Geometry check sheet. Reference: the model listing, model coordinates, mm. A direction names the side the tool comes from. Give positions to 0.01 mm unless a question says otherwise; leave off trailing zeros. Loops run counter-clockwise (first coordinate to the right, second up) from the corner with the lowest first, then second, coordinate; pieces in that order, holes last.
1. Cross-section at B-B, the plane x = 8.5. Record the cut outline in (y, z), plus the area to 3 significant figures.
2. Cross-section at C-C, the plane y = 48.5. Record the cut outline in (x, z).
3. Release check for a two-part mould opening along Z. For faces 1 (the flat face through (-1, 2, 67.5)), 2 (the flat face through (1, 0, 1)), 3 (the cylindrical face through (-47.165, -5.07, -41.506)) record: +Z half, -Z half, draft (parallel to the pull), parting line (faces both ways), or undercut.
4. Cross-section at D-D, the plane z = 47.5. Record the cut outline in (x, y).
5. Go/stop test with flat-tipped pins: pin 1 Ø10.5 at (x, z) = (-26, 17.5) entering from +Y; pin 2 Ø10 at (x, z) = (2.5, -49.5) entering from +Y; pin 3 Ø8 at (x, y) = (54.5, 7.5) entering from -Z; pin 4 Ø11 at (x, z) = (-47.43, 47.5) entering from -Y. Record where each tip stops, or that it passes through.
6. Tool access check on faces 4 (the flat face through (46, 3, -3)), 5 (the flat face through (-53, 0, -35)), 6 (the flat face through (-3, 26, -5)), 7 (the flat face through (27.643, -5, 1)), 8 (the flat face through (20, 10, 21)). Record the directions out of +Z, -Z, +X, -X, +Y, -Y that give a thin tool (end or side, any length) a straight path to the whole face; none if there is none.
7. Cross-section at A-A, the plane z = -47.5. Record the cut outline in (x, y).
8. Material ranges on L1, parallel to X at y = -4, z = -47; L2, parallel to X at y = 58, z = -33; L3, parallel to Y at x = 38, z = -35, recorded low to high.
from build123d import *

# Parameters (mm, degrees)
BASE_PLATE_SKETCH_W     = 135
BASE_PLATE_SKETCH_H     = 20
BASE_PLATE_DEPTH        = 67.5
BOTTOM_CHANNEL_DEPTH    = 152.265495074
TOP_RECESS_SKETCH_W     = 30
TOP_RECESS_SKETCH_H     = 10
TOP_RECESS_DEPTH        = 152.265495074
UPRIGHT_LUG_SKETCH_R    = 10
UPRIGHT_LUG_DEPTH       = 75
SIDE_GUSSET_DEPTH       = 3
CENTRE_START            = -37.5
CENTRE_RIB_DEPTH        = 3
MOUNTING_HOLES_SKETCH_R = 6
MOUNTING_HOLES_12_DEPTH = 128.818230312


with BuildPart() as part:
    # Base Plate Sketch → Base Plate (new, symmetric)
    with BuildSketch(Plane.XY):
        Rectangle(BASE_PLATE_SKETCH_W, BASE_PLATE_SKETCH_H)
    extrude(amount=BASE_PLATE_DEPTH, both=True)

    # Bottom Channel Sketch → Bottom Channel (cut, through all)
    with BuildSketch(Plane.XY.offset(67.5)):
        Polygon((27.643184154, 0), (0, 0), (-27.356815846, 0), (-27.356815846, -10), (27.643184154, -10), align=None)
    extrude(amount=-BOTTOM_CHANNEL_DEPTH, mode=Mode.SUBTRACT)

    # Top Recess Sketch → Top Recess (cut, through all)
    with BuildSketch(Plane.XY.offset(67.5)):
        with Locations((-52.5, 5)):
            Rectangle(TOP_RECESS_SKETCH_W, TOP_RECESS_SKETCH_H)
        with Locations((52.5, 5)):
            Rectangle(TOP_RECESS_SKETCH_W, TOP_RECESS_SKETCH_H)
    extrude(amount=-TOP_RECESS_DEPTH, mode=Mode.SUBTRACT)

    # Upright Lug Sketch → Upright Lug (add)
    with BuildSketch(Plane(origin=(37.5, 0, 0), x_dir=(0, 0, -1), z_dir=(1, 0, 0))):
        with BuildLine():
            Line((67.5, 10), (67.5, 55))
            ThreePointArc((67.5, 55), (47.5, 75), (27.5, 55))
            Line((27.5, 55), (27.5, 10))
            Line((27.5, 10), (67.5, 10))
        make_face()
        with Locations((47.5, 55)):
            Circle(UPRIGHT_LUG_SKETCH_R, mode=Mode.SUBTRACT)
    extrude(amount=-UPRIGHT_LUG_DEPTH)

    # Side Gusset Sketch → Side Gusset (add, symmetric)
    with BuildSketch(Plane.XY):
        Polygon((-67.5, 0), (-37.5, 10), (-37.5, 0), align=None)
    side_gusset = extrude(amount=SIDE_GUSSET_DEPTH, both=True)

    # Side Gusset Mirror: Side Gusset across plane
    add(side_gusset.mirror(Plane(origin=(0, 0, 0), x_dir=(0, 0, 1), z_dir=(1, 0, 0))))

    # Centre Rib Sketch → Centre Rib (add, symmetric)
    with BuildSketch(Plane(origin=(37.5, 0, 0), x_dir=(0, 0, -1), z_dir=(1, 0, 0)).offset(CENTRE_START)):
        Polygon((-67.5, 10), (35.500032612, 69.198001073), (35.500032612, 10), (29.449687004, 10), align=None)
    extrude(amount=CENTRE_RIB_DEPTH, both=True)

    # Mounting Holes Sketch → Mounting Holes Ø12 (cut, through all)
    with BuildSketch(Plane.XZ.offset(10)):
        with Locations(Location((47.571592077, -47.5, 0), (0, 0, 270))):
            Circle(MOUNTING_HOLES_SKETCH_R)
        with Locations(Location((-47.428407923, -47.5, 0), (0, 0, 270))):
            Circle(MOUNTING_HOLES_SKETCH_R)
        with Locations(Location((-47.428407923, 47.5, 0), (0, 0, 270))):
            Circle(MOUNTING_HOLES_SKETCH_R)
        with Locations(Location((47.571592077, 47.5, 0), (0, 0, 270))):
            Circle(MOUNTING_HOLES_SKETCH_R)
    extrude(amount=-MOUNTING_HOLES_12_DEPTH, mode=Mode.SUBTRACT)


solid = part.part
Result:
1. outline: (0, -67.5) - (55, -67.5) arc R20 ccw to (55, -27.5) - (10, -27.5) - (10, 67.5) - (0, 67.5) - close; hole circle Ø20 at (55, -47.5)
1. area: 3,460 mm2
2. outline: (-37.5, -67.5) - (37.5, -67.5) - (37.5, -55.1) - (-37.5, -55.1) - close; (-37.5, -39.9) - (37.5, -39.9) - (37.5, -27.5) - (3, -27.5) - (3, 0.51) - (-3, 0.51) - (-3, -27.5) - (-37.5, -27.5) - close
3. face 1: +Z half
3. face 2: draft
3. face 3: undercut
4. outline: (-67.5, -10) - (-53.43, -10) - (-53.43, 0) - (-67.5, 0) - close; (-41.43, -10) - (-27.36, -10) - (-27.36, 0) - (27.64, 0) - (27.64, -10) - (41.57, -10) - (41.57, 0) - (37.5, 0) - (37.5, 10) - (3, 10) - (3, 21.49) - (-3, 21.49) - (-3, 10) - (-37.5, 10) - (-37.5, 0) - (-41.43, 0) - close; (53.57, -10) - (67.5, -10) - (67.5, 0) - (53.57, 0) - close
5. pin 1: stops at y = 10
5. pin 2: stops at y = 75
5. pin 3: stops at z = -3
5. pin 4: passes through
6. face 4: -Z, +X, +Y
6. face 5: -Z, -X, +Y
6. face 6: +Z, -X, +Y
6. face 7: +Z, -Z, -Y
6. face 8: +Z, +X, +Y
7. outline: (-67.5, -10) - (-53.43, -10) - (-53.43, 0) - (-67.5, 0) - close; (-41.43, -10) - (-27.36, -10) - (-27.36, 0) - (27.64, 0) - (27.64, -10) - (41.57, -10) - (41.57, 0) - (37.5, 0) - (37.5, 45) - (-37.5, 45) - (-37.5, 0) - (-41.43, 0) - close; (-37.5, 65) - (37.5, 65) - (37.5, 75) - (-37.5, 75) - close; (53.57, -10) - (67.5, -10) - (67.5, 0) - (53.57, 0) - close
8. L1: x = -67.5 to -53.41, -41.45 to -27.36, 27.64 to 41.59, 53.55 to 67.5
8. L2: x = -37.5 to 37.5
8. L3: y = -10 to 0
